CAD build for the part. Positions are in the model's coordinates, mm. A direction names the side the tool comes from. Give positions to 0.01 mm unless a question says otherwise; leave off trailing zeros. Order: outer loops, then holes, each group sorted by start corner. A loop starts at its lowest first (then second) coordinate and runs counter-clockwise, first axis right, second up.
```python
from build123d import *

# Parameters (mm, degrees)
REVOLVE1_ANGLE = 10


with BuildPart() as part:
    # Sketch1 → Revolve1 (revolve, symmetric)
    with BuildSketch(Plane.XY) as revolve1_sk:
        Polygon((-109.954236571, 39.405686592), (-109.954236571, 31.426003585), (-108, 31.426003585), (-108, 10.794907178), (-109.954236571, 10.794907178), (-109.954236571, 29.163164129), (-111.581862319, 29.163164129), (-111.581862319, 39.405686592), align=None)
    revolve(axis=Axis((0, 0, 0), (-1, 0, 0)), revolution_arc=REVOLVE1_ANGLE / 2)
    revolve(revolve1_sk.sketch, axis=Axis((0, 0, 0), (1, 0, 0)), revolution_arc=REVOLVE1_ANGLE / 2)


solid = part.part
```
Item 1: Slice it at D-D (z = -0.5). Give the cut face in (x, y), and give its area (3 significant figures).
Item 2: Drop flat-ended pins along their axis: pin 1 Ø2.5 at (y, z) = (18, -0.5) entering from -X; pin 2 Ø3.5 at (y, z) = (33.5, -1) entering from +X; pin 3 Ø2 at (x, y) = (-109, 19.5) entering from -Z. Give the stop position or say it passes through.
Item 3: Slice it at B-B (y = 34.25). Give the cut face in (x, z).
Item 4: Tool access for faces 1 (the face through (-111.582, 34, 0)), 2 (the face through (-109.954, 22, 0)): list every direction of +Z, -Z, +X, -X, +Y, -Y with a clear straight run to the whole face (end or side of a thin tool).
Item 5: Two-plate mould, pull along Z, no slides. Class faces 3 (the face through (-108.963, 31.426, -0.038)), 4 (the face through (-109.954, 35, 0)), 5 (the face through (-109.368, 25.204, -2.205)), 6 (the face through (-110.779, 29.163, -0.036)): released by +Z, released by -Z, zero draft, split by the parting line, or undercut.
Item 6: Slice it at C-C (x = -109.6). Give the cut face in (y, z).
Item 7: Wall check: L1, parallel to X at y = 38, z = 1.75; L2, parallel to X at y = 26, z = 0.5; L3, parallel to Y at x = -110.45, z = 0.5. Give the ranges that are in metal, low to high.
Item 8: Slice it at A-A (z = -2). Give the cut face in (x, y), and give its area (3 significant figures).
A:
1. outline: (-111.58, 29.16) - (-109.95, 29.16) - (-109.95, 10.78) - (-108, 10.78) - (-108, 31.42) - (-109.95, 31.42) - (-109.95, 39.4) - (-111.58, 39.4) - close
1. area: 57.0 mm2
2. pin 1: stops at x = -109.95
2. pin 2: stops at x = -109.95
2. pin 3: stops at z = -1.79
3. outline: (-111.58, -3) - (-109.95, -3) - (-109.95, 3) - (-111.58, 3) - close
4. face 1: +Z, -Z, -X, +Y, -Y
4. face 2: +Z, -Z, -X, -Y
5. face 3: split by the parting line
5. face 4: zero draft
5. face 5: released by -Z
5. face 6: undercut
6. outline: (10.75, -0.94) - (31.31, -2.74) arc R31.43 ccw to (31.31, 2.74) - (10.75, 0.94) arc R10.79 cw to start
7. L1: x = -111.58 to -109.95
7. L2: x = -109.95 to -108
7. L3: y = 29.16 to 39.4
8. outline: (-111.58, 29.09) - (-109.95, 29.09) - (-109.95, 22.86) - (-108, 22.86) - (-108, 31.36) - (-109.95, 31.36) - (-109.95, 39.35) - (-111.58, 39.35) - close
8. area: 33.3 mm2
